from build123d import *

# Parameters (mm, degrees)
SKETCH_1_R          = 7.5
EXTRUDE_1_DEPTH     = 30
SKETCH_2_OUTSIDE_W  = 29.728
SKETCH_2_OUTSIDE_H  = 29.728
SKETCH_2_OUTSIDE_R  = 6
CUT_EXTRUDE_1_DEPTH = 10
CHAMFER_1_SIZE      = 0.5
SKETCH_3_W          = 1.1
SKETCH_3_H          = 0.35


with BuildPart() as part:
    # 草图1 → 凸台-拉伸1 (new, symmetric)
    with BuildSketch(Plane(origin=(0, 0, 0), x_dir=(0, 0, -1), z_dir=(1, 0, 0))):
        Circle(SKETCH_1_R)
    extrude(amount=EXTRUDE_1_DEPTH, both=True)

    # 草图2 outside → 切除-拉伸1 (cut)
    with BuildSketch(Plane(origin=(30, 0, 0), x_dir=(0, 0, -1), z_dir=(1, 0, 0))):
        Rectangle(SKETCH_2_OUTSIDE_W, SKETCH_2_OUTSIDE_H)
        Circle(SKETCH_2_OUTSIDE_R, mode=Mode.SUBTRACT)
    cut_extrude_1 = extrude(amount=-CUT_EXTRUDE_1_DEPTH, mode=Mode.SUBTRACT)

    # 镜向1: 切除-拉伸1 across plane
    add(cut_extrude_1.mirror(Plane(origin=(0, 0, 0), x_dir=(0, 0, 1), z_dir=(1, 0, 0))), mode=Mode.SUBTRACT)

    # 倒角1
    chamfer_1_edges = [part.edges().sort_by_distance(p)[0] for p in [
        (30, 0, 6),
        (-30, 0, 6),
        (-20, 0, 7.5),
        (20, 0, 7.5),
    ]]
    chamfer(chamfer_1_edges, length=CHAMFER_1_SIZE)

    # 草图3 → 切除-旋转1 (revolve, cut)
    with BuildSketch(Plane.XY, mode=Mode.PRIVATE) as cut_revolve_1_sk:
        with Locations((-18.05, -7.325)):
            Rectangle(SKETCH_3_W, SKETCH_3_H)
    cut_revolve_1 = revolve(cut_revolve_1_sk.sketch.rotate(Axis((-31.365791293, 0, 0), (1, 0, 0)), 270), axis=Axis((-31.365791293, 0, 0), (1, 0, 0)), mode=Mode.SUBTRACT)

    # 镜向2: 切除-旋转1 across plane
    add(cut_revolve_1.mirror(Plane(origin=(0, 0, 0), x_dir=(0, 0, 1), z_dir=(1, 0, 0))), mode=Mode.SUBTRACT)


solid = part.part
Read the model definition and answer for the solid it produces. Units are mm, in the model's axes. A direction names the side the tool comes from. Coordinates: 2 decimals unless noted, no trailing zeros. Loops run counter-clockwise (first coordinate to the right, second up) from the corner with the lowest first, then second, coordinate; pieces in that order, holes last.
Q1. Which of the six approach directions +Z, -Z, +X, -X, +Y, -Y give full straight-line access (tool end or side, diameter ignored) to faces 1 (the face through (-19.044, 0.33, 7.493)), 2 (the face through (30, 0, 0)), 3 (the face through (-20, 2, -6)), 4 (the face through (18.04, -7.09, -0.93)), 5 (the face through (25, 0, 6))?
Q2. The part is cut by section A-A on x = 12. Write down the section's boundary in (y, z).
Q3. Consider probe 1 along Z at (x, y) = (-7, 0.25); probe 2 along Y at (x, z) = (-18, -1.5); probe 3 along Y at (x, z) = (-19.5, 4.25). Determine where each line is inside the solid, lowest interval first.
Q4. Each of these flat-tipped pins is pushed along its axis until it touches: pin 1 Ø4 at (x, z) = (23.5, -3.5) entering from -Y; pin 2 Ø8 at (x, y) = (11, 5.5) entering from +Z; pin 3 Ø8 at (x, y) = (-11.5, -5.5) entering from -Z. Where does it stop, or does it pass through?
Q5. The mould has two halves that part along X. Classify faces 6 (the face through (19.056, 0.33, 7.493)), 7 (the face through (-18.04, -7.09, -0.93)), 8 (the face through (20, 2, -6)), 9 (the face through (-30, 0, 0)): +X half, -X half, draft (parallel to the pull), parting line (faces both ways), or undercut.
Results below:
1. face 1: +X, -X
1. face 2: +Z, -Z, +X, +Y, -Y
1. face 3: -X
1. face 4: none
1. face 5: +X
2. outline: circle Ø15 at (0, 0)
3. probe 1: z = -7.5 to 7.5
3. probe 2: y = -6.99 to 6.99
3. probe 3: y = -6.18 to 6.18
4. pin 1: stops at y = -5.81
4. pin 2: stops at z = 7.35
4. pin 3: stops at z = -7.35
5. face 6: draft
5. face 7: undercut
5. face 8: +X half
5. face 9: -X half
